Read the model definition and answer for the solid it produces. Units are mm, in the model's axes. Coordinates: 2 decimals unless noted, no trailing zeros. Write each loop counter-clockwise with the first axis right and the second up, starting at its lowest first coordinate (ties: lowest second). Pieces come first, ordered by that corner, then holes. Notation, with made-up numbers: (75, -33.75) -> (130, -33.75) arc R29 cw to (130, -9.75) -> close; hole circle Ø5 at (-20, -18.5). An arc over 180 degrees is marked (long way). Answer in a Markdown table with one row per item. Add a question column.
Item 1: Given pin 1 Ø4 at (x, z) = (8, -20) entering from -Y, flat-ended and moving along its own axis, determine where the tip first touches the part or whether it passes through.
Item 2: Section B-B on z = -20 is taken. Write down the section's boundary in (x, y), then the cut area to 3 significant figures.
Item 3: Straight lines are drawn through the part: line 1 (X direction, y = 0.6, z = -20); line 2 (Z direction, x = -7, y = 0.9); line 3 (X direction, y = 0.1, z = 31.5). For each, find the intervals that lie inside material, in ascending order. Write a range as from..to.
Item 4: Section A-A on y = 1.45 is taken. Write down the section's boundary in (x, z).
Item 5: Section C-C on x = -8 is taken. Write down the section's boundary in (y, z).
Item 6: Section D-D on x = 2.5 is taken. Write down the section's boundary in (y, z).
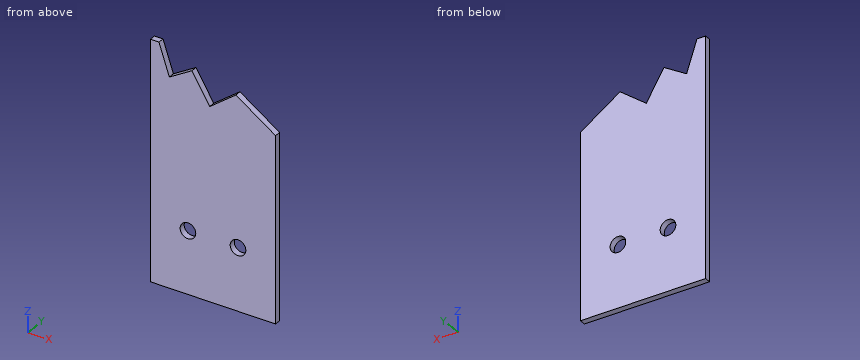
```python
from build123d import *

# Parameters (mm, degrees)
SKETCH1_W           = 40
SKETCH1_H           = 80
BOSS_EXTRUDE1_DEPTH = 2
SKETCH2_R           = 2.5
CUT_EXTRUDE1_DEPTH  = 10
CUT_EXTRUDE2_DEPTH  = 10


with BuildPart() as part:
    # Sketch1 → Boss-Extrude1 (new body)
    with BuildSketch(Plane(origin=(0, 0, 0), x_dir=(1, 0, 0), z_dir=(0, 1, 0))):
        Rectangle(SKETCH1_W, SKETCH1_H)
    extrude(amount=BOSS_EXTRUDE1_DEPTH)

    # Sketch2 → Cut-Extrude1 (cut)
    with BuildSketch(Plane.XZ):
        with Locations(Location((8, -20, 0), (0, 0, 270))):
            Circle(SKETCH2_R)
        with Locations(Location((-8, -20, 0), (0, 0, 270))):
            Circle(SKETCH2_R)
    extrude(amount=-CUT_EXTRUDE1_DEPTH, mode=Mode.SUBTRACT)

    # Sketch3 → Cut-Extrude2 (cut)
    with BuildSketch(Plane(origin=(0, 2, 0), x_dir=(1, 0, 0), z_dir=(0, 1, 0))):
        Polygon((20, -19.19837027), (7.322915473, -27.754938711), (-1.053514684, -21.360029666), (-6.727870598, -30.72722038), (-13.940955905, -26.357755241), (-17.265960151, -36.22143801), (-20, -36.22143801), (-20, -40), (20, -40), align=None)
    extrude(amount=-CUT_EXTRUDE2_DEPTH, mode=Mode.SUBTRACT)


solid = part.part
```
Results below:
| question | item | result |
|---|---|---|
| 1 | pin 1 | passes through |
| 2 | outline | (-20, 0) -> (-10.5, 0) -> (-10.5, 2) -> (-20, 2) -> close; (-5.5, 0) -> (5.5, 0) -> (5.5, 2) -> (-5.5, 2) -> close; (10.5, 0) -> (20, 0) -> (20, 2) -> (10.5, 2) -> close |
| 2 | area | 60.0 mm2 |
| 3 | line 1 | x = -20..-10.5, -5.5..5.5, 10.5..20 |
| 3 | line 2 | z = -40..-22.29, -17.71..30.56 |
| 3 | line 3 | x = -20..-15.67 |
| 4 | outline | (-20, -40) -> (20, -40) -> (20, 19.2) -> (7.32, 27.75) -> (-1.05, 21.36) -> (-6.73, 30.73) -> (-13.94, 26.36) -> (-17.27, 36.22) -> (-20, 36.22) -> close; hole circle Ø5 at (-8, -20); hole circle Ø5 at (8, -20) |
| 5 | outline | (0, -40) -> (2, -40) -> (2, -22.5) -> (0, -22.5) -> close; (0, -17.5) -> (2, -17.5) -> (2, 29.96) -> (0, 29.96) -> close |
| 6 | outline | (0, -40) -> (2, -40) -> (2, 24.07) -> (0, 24.07) -> close |
